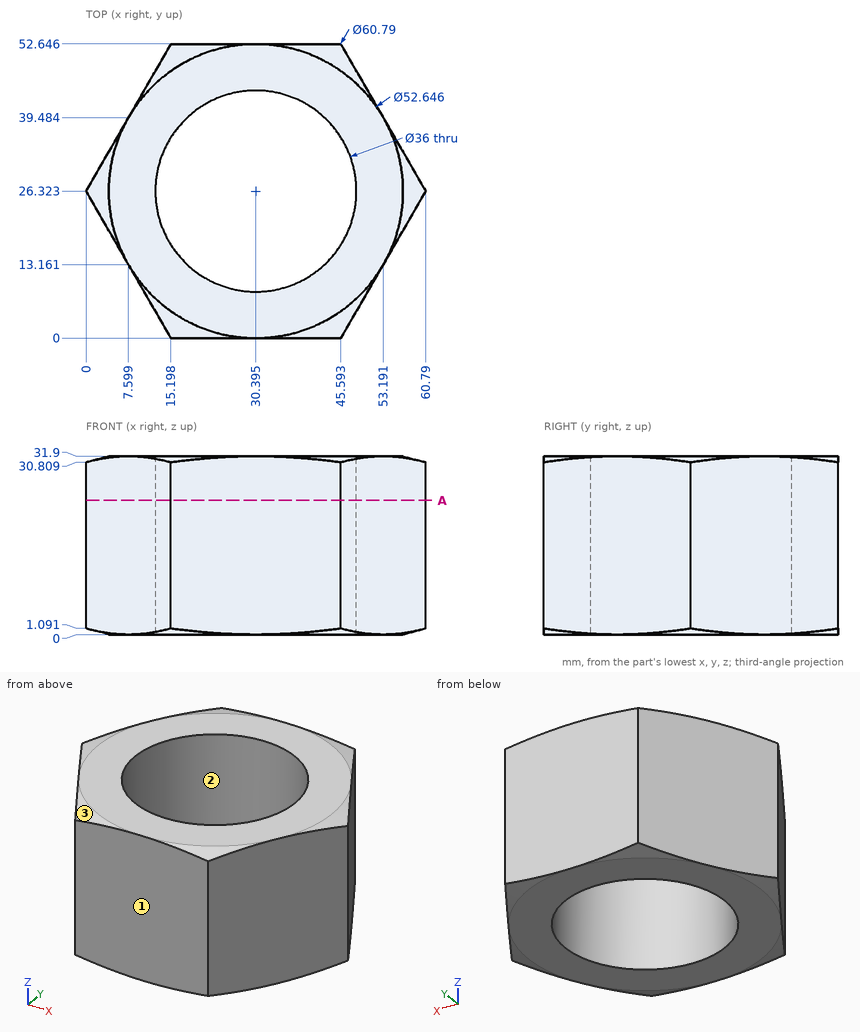
Input: dimensioned drawing with shaded views. Units: mm. Origin: part minimum x, y, z. Give positions to 0.01 mm unless a question says otherwise; leave off trailing zeros. Write each loop counter-clockwise with the first axis right and the second up, starting at its lowest first coordinate (ties: lowest second). Pieces come first, ordered by that corner, then holes.
1. Pin query (flat end, axial travel): P1, Ø6, axis at x = 18.5, y = 21.5, coming from the -Z side; P2, Ø6, axis at y = 39.5, z = 11, coming from the +X side (1 decimal); P3, Ø4, axis at x = 10, z = 27.5, coming from the -Y side; P4, Ø6, axis at y = 21, z = 4, coming from the +X side. Return the tip coordinate at first contact, or that it passes through.
2. Section query A-A, the plane z = 24. Return loops of the section in (x, y) (1 decimal), then the cut area to 3 significant figures.
3. Line query: probe 1 along Y at (x, z) = (30, 7) (1 decimal); probe 2 along Y at (x, z) = (14.5, 25.5) (1 decimal); probe 3 along X at (y, z) = (39, 12) (1 decimal). Output: solid intervals per line, ascending.
4. Draft query along X for the marked faces 1, 2 and 3. Return one class per face: released by +X, released by -X, zero draft, split by the parting line, or undercut.
Computed:
1. P1: passes through
1. P2: stops at x = 54.9
1. P3: stops at y = 5.54
1. P4: stops at x = 59.45
2. outline: (0, 26.3) - (15.2, 0) - (45.6, 0) - (60.8, 26.3) - (45.6, 52.6) - (15.2, 52.6) - close; hole circle Ø36 at (30.4, 26.3)
2. area: 1,380 mm2
3. probe 1: y = 0 to 8.3, 44.3 to 52.6
3. probe 2: y = 1.2 to 17.9, 34.8 to 51.4
3. probe 3: x = 7.3 to 17.6, 43.2 to 53.5
4. face 1: zero draft
4. face 2: undercut
4. face 3: released by -X
